Input: part model. Units: mm. Frame: model coordinates. Face numbers are marked on the shaded views. A direction names the side the tool comes from. Coordinates: 2 decimals unless noted, no trailing zeros. Write each loop counter-clockwise with the first axis right and the second up, starting at its lowest first coordinate (ties: lowest second). Pieces come first, ordered by that corner, then holes.
1) Pin query (flat end, axial travel): pin 1 Ø1.5 at (x, y) = (25.5, 50.5) entering from +Z; pin 2 Ø2 at (y, z) = (54.5, -56) entering from +X; pin 3 Ø12 at (y, z) = (28.5, -75) entering from +X. Return the tip coordinate at first contact, or that it passes through.
2) Section query C-C (z = 5.5). Output: boundary loops of the cut face in (x, y), then the cut area to 3 significant figures.
3) Set-up query: the marked faces 1, 2 and 3. Return all of +Z, -Z, +X, -X, +Y, -Y with unobstructed straight access to the full face (end or side cutting, diameter ignored); none if empty.
4) Section query D-D (z = 26.5). Output: boundary loops of the cut face in (x, y).
5) Line query: L1, parallel to Y at x = 74, z = 2; L2, parallel to Z at x = 14, y = 33.5; L3, parallel to Z at x = 72, y = 6. Output: solid intervals per line, ascending.
6) Section query A-A (x = 40). Output: boundary loops of the cut face in (y, z), then the cut area to 3 significant figures.
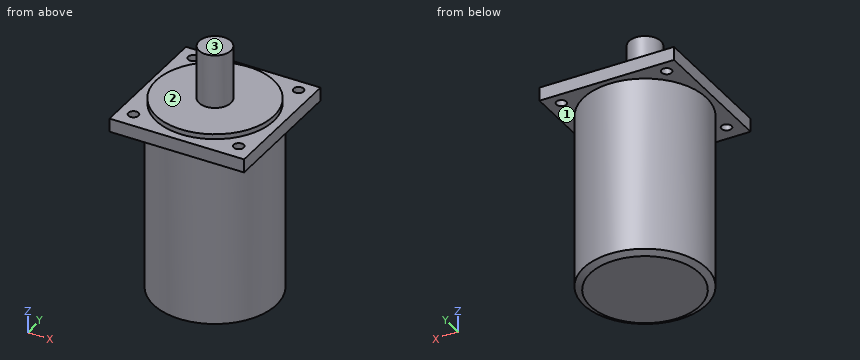
from build123d import *

# Parameters (mm, degrees)
SKETCH_1_W          = 80
SKETCH_1_H          = 80
EXTRUDE_1_DEPTH     = 8
SKETCH_2_R          = 35
EXTRUDE_2_DEPTH     = 3
SKETCH_3_R          = 9.5
EXTRUDE_3_DEPTH     = 32
SKETCH_4_R          = 36.492471365
EXTRUDE_4_DEPTH     = 106
CUT_EXTRUDE_1_REACH = 162.611
SKETCH_5_R          = 3
CHAMFER_1_SIZE      = 2
CHAMFER_1_SIZE2     = 4


with BuildPart() as part:
    # 草图1 → 拉伸1 (new body)
    with BuildSketch(Plane.XY):
        with Locations((40, 40)):
            Rectangle(SKETCH_1_W, SKETCH_1_H)
    extrude(amount=EXTRUDE_1_DEPTH)

    # 草图2 → 拉伸2 (add)
    with BuildSketch(Plane.XY.offset(8)):
        with Locations(Location((40, 40, 0), (0, 0, 180))):
            Circle(SKETCH_2_R)
    extrude(amount=EXTRUDE_2_DEPTH)

    # 草图3 → 拉伸3 (add)
    with BuildSketch(Plane.XY.offset(11)):
        with Locations((40, 40)):
            Circle(SKETCH_3_R)
    extrude(amount=EXTRUDE_3_DEPTH)

    # 草图4 → 拉伸4 (add)
    with BuildSketch(Plane(origin=(0, 0, 0), x_dir=(-1, 0, 0), z_dir=(0, 0, -1))):
        with Locations((-40, 40)):
            Circle(SKETCH_4_R)
    extrude(amount=EXTRUDE_4_DEPTH)

    # 草图5 → 切除-拉伸1 (cut, up to next)
    with BuildSketch(Plane.XY.offset(8), mode=Mode.PRIVATE) as cut_extrude_1_sk1:
        with Locations((8.713677805, 72.344490157)):
            Circle(SKETCH_5_R)
    cut_extrude_1_tool1 = extrude(cut_extrude_1_sk1.sketch, amount=-CUT_EXTRUDE_1_REACH, mode=Mode.PRIVATE) & part.part
    # 草图5 → 切除-拉伸1 (cut, up to next)
    with BuildSketch(Plane.XY.offset(8), mode=Mode.PRIVATE) as cut_extrude_1_sk2:
        with Locations((71.286322195, 72.344490157)):
            Circle(SKETCH_5_R)
    cut_extrude_1_tool2 = extrude(cut_extrude_1_sk2.sketch, amount=-CUT_EXTRUDE_1_REACH, mode=Mode.PRIVATE) & part.part
    # 草图5 → 切除-拉伸1 (cut, up to next)
    with BuildSketch(Plane.XY.offset(8), mode=Mode.PRIVATE) as cut_extrude_1_sk3:
        with Locations((71.286322195, 9.771845767)):
            Circle(SKETCH_5_R)
    cut_extrude_1_tool3 = extrude(cut_extrude_1_sk3.sketch, amount=-CUT_EXTRUDE_1_REACH, mode=Mode.PRIVATE) & part.part
    # 草图5 → 切除-拉伸1 (cut, up to next)
    with BuildSketch(Plane.XY.offset(8), mode=Mode.PRIVATE) as cut_extrude_1_sk4:
        with Locations((8.713677805, 9.771845767)):
            Circle(SKETCH_5_R)
    cut_extrude_1_tool4 = extrude(cut_extrude_1_sk4.sketch, amount=-CUT_EXTRUDE_1_REACH, mode=Mode.PRIVATE) & part.part
    add(cut_extrude_1_tool1.solids().sort_by_distance((8.713678, 72.34449, 8))[0], mode=Mode.SUBTRACT)
    add(cut_extrude_1_tool2.solids().sort_by_distance((71.286322, 72.34449, 8))[0], mode=Mode.SUBTRACT)
    add(cut_extrude_1_tool3.solids().sort_by_distance((71.286322, 9.771846, 8))[0], mode=Mode.SUBTRACT)
    add(cut_extrude_1_tool4.solids().sort_by_distance((8.713678, 9.771846, 8))[0], mode=Mode.SUBTRACT)

    # 倒角1
    chamfer_1_edges = [part.edges().sort_by_distance(p)[0] for p in [
        (76.492471365, 40, -106),
    ]]
    chamfer_1_side = [part.faces().sort_by_distance(p)[0] for p in [
        (76.492471365, 40, -53),
    ]]
    chamfer(chamfer_1_edges, length=CHAMFER_1_SIZE, length2=CHAMFER_1_SIZE2, reference=chamfer_1_side[0])


solid = part.part
Answer:
1. pin 1: stops at z = 11
1. pin 2: stops at x = 73.9
1. pin 3: stops at x = 76.08
2. outline: (0, 0) - (80, 0) - (80, 80) - (0, 80) - close; hole circle Ø6 at (8.71, 9.77); hole circle Ø6 at (8.71, 72.34); hole circle Ø6 at (71.29, 9.77); hole circle Ø6 at (71.29, 72.34)
2. area: 6,290 mm2
3. face 1: -Z
3. face 2: +Z
3. face 3: +Z, +X, -X, +Y, -Y
4. outline: circle Ø19 at (40, 40)
5. L1: y = 0 to 8.49, 11.05 to 71.07, 73.62 to 80
5. L2: z = -106 to 11
5. L3: z = 0 to 8
6. outline: (0, 0) - (3.51, 0) - (3.51, -104) - (7.51, -106) - (72.49, -106) - (76.49, -104) - (76.49, 0) - (80, 0) - (80, 8) - (75, 8) - (75, 11) - (49.5, 11) - (49.5, 43) - (30.5, 43) - (30.5, 11) - (5, 11) - (5, 8) - (0, 8) - close
6. area: 9,190 mm2
